Read the model definition and answer for the solid it produces. Units are mm, in the model's axes. A direction names the side the tool comes from. Coordinates: 2 decimals unless noted, no trailing zeros. Loops run counter-clockwise (first coordinate to the right, second up) from the corner with the lowest first, then second, coordinate; pieces in that order, holes last. Notation, with made-up numbers: (29, 78) -> (78, 78) arc R8 ccw to (78, 85) -> close; hole circle Ø9 at (-23.75, 40.25). An arc over 180 degrees is marked (long way). Answer as a JSON object with one key per item and string values. Group by question number.
Q1. The part is cut by section D-D on y = 2.25. Write down the section's boundary in (x, z), and give its area (3 significant figures).
Q2. For faces 1 (the cylindrical face through (0.54, -2.44, -7.99)), 2 (the flat face through (3, -1, 0)), 3 (the cylindrical face through (-5.158, -3.955, 2.465)), 4 (the cylindrical face through (0, -2, 6)), determine the directions among +Z, -Z, +X, -X, +Y, -Y from which every point of the face is accessible in a straight line to the end or side of a thin tool.
Q3. Straight lines are drawn through the part: line 1 along Z through (x, y) = (1.5, 2.5); line 2 along Z through (x, y) = (-2.25, 5); line 3 along Z through (x, y) = (2.25, -0.5). For each, find the intervals that lie inside material, in ascending order. Write a range as [from, to].
Q4. The part is cut by section C-C on z = -5.5. Write down the section's boundary in (x, y).
Q5. The part is cut by section A-A on y = 0. Write down the section's boundary in (x, z).
Q6. Each of these flat-tipped pins is pushed along its axis until it touches: P1, Ø4, axis at x = -3.5, z = -5, coming from the -Y side; P2, Ø6, axis at x = 3.5, z = 4, coming from the +Y side. Where does it stop, or does it pass through?
Q7. Determine the mould class of faces 5 (the flat face through (0, 0, 7)), 6 (the flat face through (0, 0, -10)), 7 (the flat face through (-2, -2, -8.5)) for opening direction Z: released by +Z, released by -Z, zero draft, split by the parting line, or undercut.
from build123d import *

# Parameters (mm, degrees)
SKETCH1_R      = 6.5
EXTRUDE1_DEPTH = 5
SKETCH2_R      = 2
EXTRUDE2_DEPTH = 2
SKETCH3_R      = 3
EXTRUDE3_DEPTH = 7.5
SKETCH4_R      = 2.5
EXTRUDE5_DEPTH = 1
SKETCH6_R      = 3
EXTRUDE6_DEPTH = 1.5


with BuildPart() as part:
    # Sketch1 → Extrude1 (new body)
    with BuildSketch(Plane.XY):
        Circle(SKETCH1_R)
    extrude(amount=EXTRUDE1_DEPTH)

    # Sketch2 → Extrude2 (add)
    with BuildSketch(Plane.XY.offset(5)):
        Circle(SKETCH2_R)
    extrude(amount=EXTRUDE2_DEPTH)

    # Sketch3 → Extrude3 (add)
    with BuildSketch(Plane(origin=(0, 0, 0), x_dir=(-1, 0, 0), z_dir=(0, 0, -1))):
        with Locations(Location((0, 0, 0), (0, 0, 180))):
            Circle(SKETCH3_R)
    extrude(amount=EXTRUDE3_DEPTH)

    # Sketch4 → Extrude5 (add)
    with BuildSketch(Plane(origin=(0, 0, -7.5), x_dir=(-1, 0, 0), z_dir=(0, 0, -1))):
        Circle(SKETCH4_R)
    extrude(amount=EXTRUDE5_DEPTH)

    # Sketch6 → Extrude6 (add)
    with BuildSketch(Plane(origin=(0, 0, -8.5), x_dir=(-1, 0, 0), z_dir=(0, 0, -1))):
        with Locations(Location((0, 0, 0), (0, 0, 180))):
            Circle(SKETCH6_R)
    extrude(amount=EXTRUDE6_DEPTH)


solid = part.part
Final values:
{
 "1": {"outline": "(-6.1, 0) -> (-1.98, 0) -> (-1.98, -7.5) -> (-1.09, -7.5) -> (-1.09, -8.5) -> (-1.98, -8.5) -> (-1.98, -10) -> (1.98, -10) -> (1.98, -8.5) -> (1.09, -8.5) -> (1.09, -7.5) -> (1.98, -7.5) -> (1.98, 0) -> (6.1, 0) -> (6.1, 5) -> (-6.1, 5) -> close", "area": "98.9 mm2"},
 "2": {"face 1": "none", "face 2": "-Z", "face 3": "+Z, -Z", "face 4": "+Z"},
 "3": {"line 1": "z = [-10, -8.5], [-7.5, 5]", "line 2": "z = [0, 5]", "line 3": "z = [-10, 5]"},
 "4": {"outline": "circle Ø6 at (0, 0)"},
 "5": {"outline": "(-6.5, 0) -> (-3, 0) -> (-3, -7.5) -> (-2.5, -7.5) -> (-2.5, -8.5) -> (-3, -8.5) -> (-3, -10) -> (3, -10) -> (3, -8.5) -> (2.5, -8.5) -> (2.5, -7.5) -> (3, -7.5) -> (3, 0) -> (6.5, 0) -> (6.5, 5) -> (2, 5) -> (2, 7) -> (-2, 7) -> (-2, 5) -> (-6.5, 5) -> close"},
 "6": {"P1": "stops at y = -2.6", "P2": "stops at y = 6.48"},
 "7": {"face 5": "released by +Z", "face 6": "released by -Z", "face 7": "undercut"}
}
